For this review, use the dimensioned drawing (mm, ordinates from the lowest corner) and the shaded views. A direction names the side the tool comes from. Give positions to 0.01 mm unless a question says otherwise; leave off trailing zeros. Loops run counter-clockwise (first coordinate to the right, second up) from the corner with the lowest first, then second, coordinate; pieces in that order, holes last. Notation, with made-up numbers: M 55.25,78.5 L 90.25,78.5 A38 cw 90.25,116.5 Z; hole C -27.5,37 d9. An arc over 180 degrees is marked long. Use a Markdown table: item, result. Add a question column.
(1) For the marked faces 1, 2, 3, 4 and 5, list the 3-axis set-ups (+Z, -Z, +X, -X, +Y, -Y) from which the entire face can be reached by the end or side of a thin tool; tool diameter is ignored.
(2) Add section B-B, the plane y = 24. Give the boundary of the cut face in (x, z).
(3) Insertion check: pin 1 Ø6 at (y, z) = (98.5, 15.5) entering from -X; pin 2 Ø12 at (x, z) = (25, 31) entering from -Y; pin 3 Ø10 at (x, z) = (36, 6.5) entering from +Y; pin 4 Ø1 at (y, z) = (69, 36) entering from -X. Each pin has a flat end and moves straight along its axis. Give the tip position at first contact, or say it passes through.
(4) For probe 1 along Y at (x, z) = (1.55, 25); probe 2 along Y at (x, z) = (4, 43); probe 3 along X at (y, z) = (85.5, 27), list the stretches that pass through material, from the lowest coordinate up.
(5) Add section D-D, the plane z = 25. Give the boundary of the cut face in (x, y).
(6) Add section C-C, the plane x = 36. Give the boundary of the cut face in (y, z), then the cut area to 3 significant figures.
(7) Add section A-A, the plane x = 22. Give the boundary of the cut face in (y, z).
(8) Draft analysis for pull direction Y (two halves, no side actions). For the marked faces 6, 7 and 8, state which applies: pulls with the +Y half, pulls with the -Y half, needs draft (parallel to the pull), parting line crosses it, or undercut.
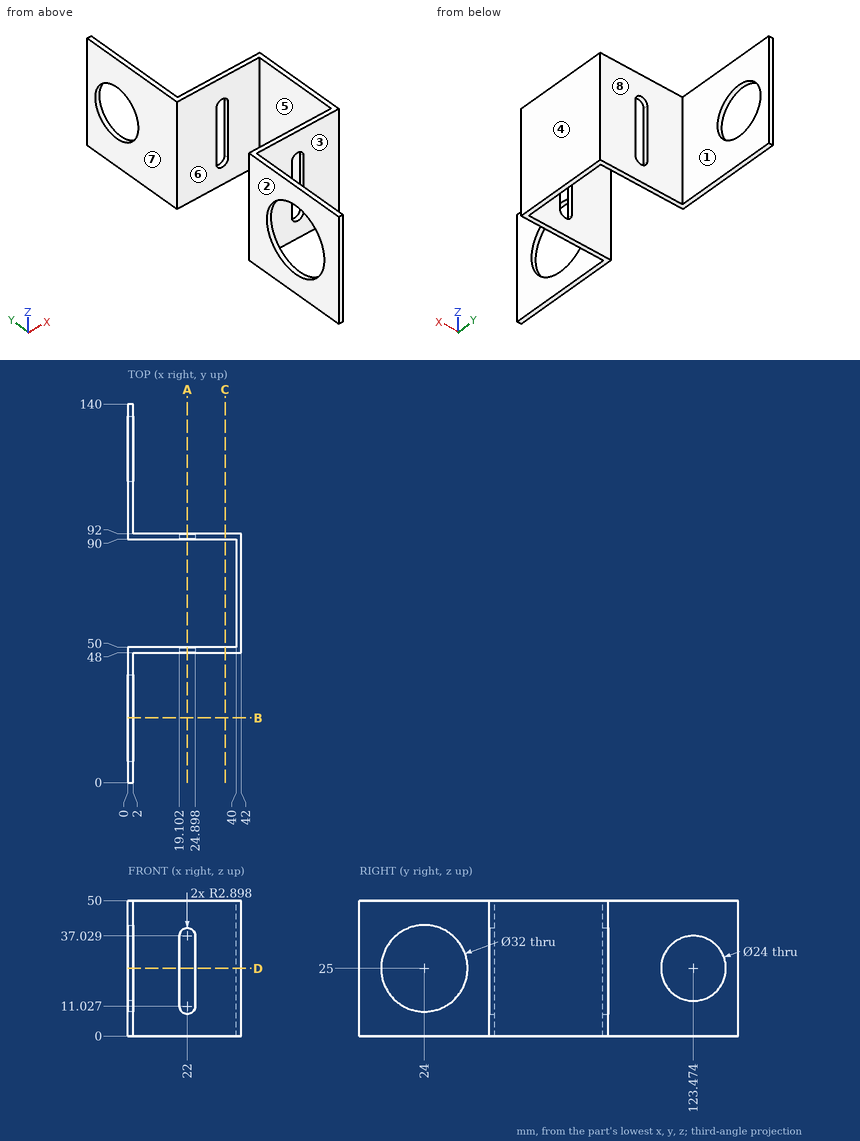
Established:
| question | item | result |
|---|---|---|
| 1 | face 1 | +Z, -Z, +X, +Y |
| 1 | face 2 | +Z, -Z, -X, +Y, -Y |
| 1 | face 3 | +Z, -Z, +X, -Y |
| 1 | face 4 | +Z, -Z, +X, +Y, -Y |
| 1 | face 5 | +Z, -Z, -X |
| 2 | outline | M 0,0 L 2,0 L 2,9 L 0,9 Z; M 0,41 L 2,41 L 2,50 L 0,50 Z |
| 3 | pin 1 | x = 0 |
| 3 | pin 2 | y = 48 |
| 3 | pin 3 | y = 92 |
| 3 | pin 4 | x = 40 |
| 4 | probe 1 | 0 to 8, 40 to 50, 90 to 111.47, 135.47 to 140 |
| 4 | probe 2 | 48 to 50, 90 to 92 |
| 4 | probe 3 | 40 to 42 |
| 5 | outline | M 0,0 L 2,0 L 2,8 L 0,8 Z; M 0,40 L 2,40 L 2,48 L 19.1,48 L 19.1,50 L 0,50 Z; M 0,90 L 19.1,90 L 19.1,92 L 2,92 L 2,111.47 L 0,111.47 Z; M 0,135.47 L 2,135.47 L 2,140 L 0,140 Z; M 24.9,48 L 42,48 L 42,92 L 24.9,92 L 24.9,90 L 40,90 L 40,50 L 24.9,50 Z |
| 6 | outline | M 48,0 L 50,0 L 50,50 L 48,50 Z; M 90,0 L 92,0 L 92,50 L 90,50 Z |
| 6 | area | 200 mm^2 |
| 7 | outline | M 48,0 L 50,0 L 50,8.13 L 48,8.13 Z; M 48,39.93 L 50,39.93 L 50,50 L 48,50 Z; M 90,0 L 92,0 L 92,8.13 L 90,8.13 Z; M 90,39.93 L 92,39.93 L 92,50 L 90,50 Z |
| 8 | face 6 | undercut |
| 8 | face 7 | needs draft |
| 8 | face 8 | pulls with the +Y half |
